from build123d import *

# Parameters (mm, degrees)
BOSS_EXTRUDE1_DEPTH = 4
SKETCH2_R           = 4
CUT_EXTRUDE2_DEPTH  = 45.634627813
SKETCH3_W           = 18
SKETCH3_H           = 4
SKETCH3_W_2         = 15
SKETCH3_H_2         = 2
CUT_EXTRUDE3_DEPTH  = 46.30176597
CHAMFER1_SIZE       = 2
CHAMFER2_SIZE       = 0.5


with BuildPart() as part:
    # Sketch1 → Boss-Extrude1 (new, symmetric)
    with BuildSketch(Plane.XY):
        with BuildLine():
            Line((-37.5, 6), (37.5, 6))
            ThreePointArc((37.5, 6), (43.5, 0), (37.5, -6))
            Line((37.5, -6), (-37.5, -6))
            ThreePointArc((-37.5, -6), (-43.5, 0), (-37.5, 6))
        make_face()
    extrude(amount=BOSS_EXTRUDE1_DEPTH, both=True)

    # Sketch2 → Cut-Extrude2 (cut, through all)
    with BuildSketch(Plane.XY.offset(4)):
        with Locations((37.5, 0)):
            Circle(SKETCH2_R)
        with Locations((-37.5, 0)):
            Circle(SKETCH2_R)
    extrude(amount=-CUT_EXTRUDE2_DEPTH, mode=Mode.SUBTRACT)

    # Sketch3 → Cut-Extrude3 (cut, through all)
    with BuildSketch(Plane(origin=(0, 6, 0), x_dir=(1, 0, 0), z_dir=(0, 1, 0))):
        with Locations((34.5, -2)):
            Rectangle(SKETCH3_W, SKETCH3_H)
        with Locations((-36, -3)):
            Rectangle(SKETCH3_W_2, SKETCH3_H_2)
        with Locations((-36, 3)):
            Rectangle(SKETCH3_W_2, SKETCH3_H_2)
    extrude(amount=-CUT_EXTRUDE3_DEPTH, mode=Mode.SUBTRACT)

    # Chamfer1
    chamfer1_edges = [part.edges().sort_by_distance(p)[0] for p in [
        (25.5, -6, 2),
        (25.5, 6, 2),
        (-28.5, 6, 3),
        (-28.5, -6, 3),
        (-28.5, -6, -3),
        (-28.5, 6, -3),
    ]]
    chamfer(chamfer1_edges, length=CHAMFER1_SIZE)

    # Chamfer2
    chamfer2_edges = [part.edges().sort_by_distance(p)[0] for p in [
        (33.5, 0, -4),
        (33.5, 0, 0),
        (-41.5, 0, 2),
        (-41.5, 0, -2),
    ]]
    chamfer(chamfer2_edges, length=CHAMFER2_SIZE)


solid = part.part
Here's how the part is built. I have some questions about the finished solid (model axes, mm). A direction names the side the tool comes from. Give positions to 0.01 mm unless a question says otherwise; leave off trailing zeros. Loops run counter-clockwise (first coordinate to the right, second up) from the corner with the lowest first, then second, coordinate; pieces in that order, holes last. Notation, with made-up numbers: (69.5, 34.5) -> (91.5, 34.5) arc R25 ccw to (91.5, 67.5) -> close; hole circle Ø8 at (83.25, 65). An arc over 180 degrees is marked (long way). Answer as a JSON object with one key per item and string values. Group by question number.
Item 1: Will these pins go through, and if not, where does the flat tip stop? pin 1 (7 mm diameter, centred on x = -37.5, y = 0, fed in from +Z); pin 2 (1 mm diameter, centred on y = -1, z = 3, fed in from -X); pin 3 (4.5 mm diameter, centred on y = -0.5, z = 1.5, fed in from +X); pin 4 (1.5 mm diameter, centred on y = 3.5, z = 2.5, fed in from -X).
Item 2: Imagine slicing it at A-A on y = 0. Write out the boundary of the cut face in (x, z).
Item 3: I need wall thicknesses on L1, parallel to Y at x = 37.5, z = -2.25; L2, parallel to X at y = -2.25, z = -1; L3, parallel to Z at x = 30, y = -5.5. Which ranges of each line are inside material? Lowest first, please.
Item 4: Thinking about a two-plate mould opening in X: for faces 1 (the flat face through (-31, 0, 2)), 2 (the flat face through (-27.5, 5, 3)), 3 (the cylindrical face through (43.5, 0.1, -2)), 4 (the cylindrical face through (34.3, -2.4, -2)), which applies, pulls with the +X half, pulls with the -X half, needs draft (parallel to the pull), parting line crosses it, or undercut?
Item 5: On a 3-axis mill with a long thin cutter (end or side, diameter ignored), from which of +Z, -Z, +X, -X, +Y, -Y can I reach the whole of each face in a straight line? I mean faces 5 (the flat face through (24.5, -5, 2)), 6 (the flat face through (-28.5, 0, -3)), 7 (the flat face through (25.5, 0, 2)). Say none if no direction works.
Item 6: Imagine slicing it at B-B on z = 0.75. Write out the boundary of the cut face in (x, y), then the cut area to 3 significant figures.
Answer list:
{
 "1": {"pin 1": "passes through", "pin 2": "stops at x = -28.5", "pin 3": "stops at x = 43.5", "pin 4": "stops at x = -42.73"},
 "2": {"outline": "(-43.5, -2) -> (-42, -2) -> (-41.5, -1.5) -> (-41.5, 1.5) -> (-42, 2) -> (-43.5, 2) -> close; (-33.5, -1.5) -> (-33, -2) -> (-28.5, -2) -> (-28.5, -4) -> (33, -4) -> (33.5, -3.5) -> (33.5, -0.5) -> (33, 0) -> (25.5, 0) -> (25.5, 4) -> (-28.5, 4) -> (-28.5, 2) -> (-33, 2) -> (-33.5, 1.5) -> close; (41.5, -3.5) -> (42, -4) -> (43.5, -4) -> (43.5, 0) -> (42, 0) -> (41.5, -0.5) -> close"},
 "3": {"L1": "y = -6 to -4, 4 to 6", "L2": "x = -43.06 to -40.81, -34.19 to 34.19, 40.81 to 43.06", "L3": "z = -4 to 0"},
 "4": {"face 1": "needs draft", "face 2": "pulls with the -X half", "face 3": "pulls with the +X half", "face 4": "undercut"},
 "5": {"face 5": "+Z, +X, -Y", "face 6": "-Z, -X, +Y, -Y", "face 7": "+Z, +X, +Y, -Y"},
 "6": {"outline": "(-37.5, -6) -> (23.5, -6) -> (25.5, -4) -> (25.5, 4) -> (23.5, 6) -> (-37.5, 6) arc R6 ccw to start; hole circle Ø8 at (-37.5, 0)", "area": "758 mm2"}
}
